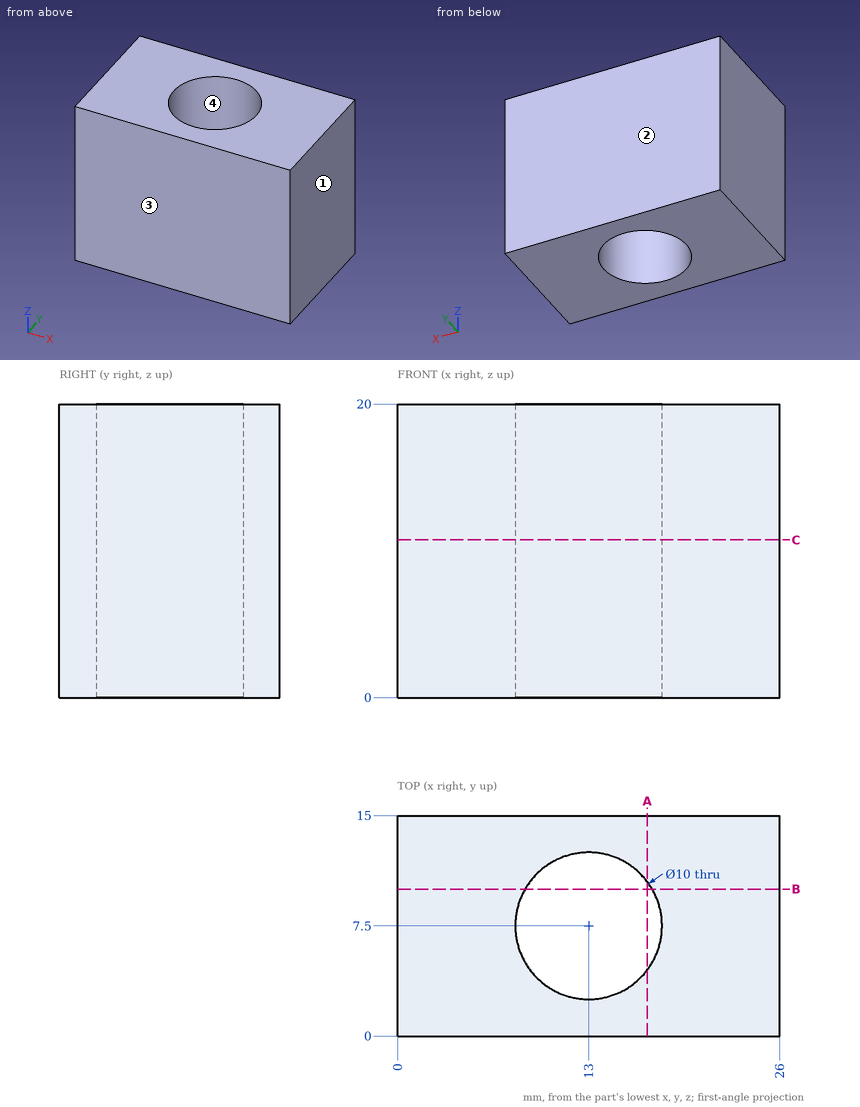
For this review, use the dimensioned drawing (mm, ordinates from the lowest corner) and the shaded views. Coordinates: 2 decimals unless noted, no trailing zeros. Loops run counter-clockwise (first coordinate to the right, second up) from the corner with the lowest first, then second, coordinate; pieces in that order, holes last. Notation, with made-up numbers: M 70,67 L 110,67 A26 ccw 110,84 Z; hole C 12.25,54 d3. An arc over 180 degrees is marked long. Answer as CSV lines item,"result".
Item 1: For probe 1 along Y at (x, z) = (13, 11.75); probe 2 along X at (y, z) = (11.25, 8); probe 3 along X at (y, z) = (9.75, 15), list the stretches that pass through material, from the lowest coordinate up.
Answer list:
probe 1,"0 to 2.5, 12.5 to 15"
probe 2,"0 to 9.69, 16.31 to 26"
probe 3,"0 to 8.53, 17.47 to 26"
Item 2: Add section C-C on z = 10.75. State the section outline as (x, y) points.
Answer list:
outline,"M 0,0 L 26,0 L 26,15 L 0,15 Z; hole C 13,7.5 d10"
Item 3: Add section A-A on x = 17. State the section outline as (y, z) points.
Answer list:
outline,"M 0,0 L 4.5,0 L 4.5,20 L 0,20 Z; M 10.5,0 L 15,0 L 15,20 L 10.5,20 Z"
Item 4: Add section B-B on y = 10. State the section outline as (x, z) points.
Answer list:
outline,"M 0,0 L 8.67,0 L 8.67,20 L 0,20 Z; M 17.33,0 L 26,0 L 26,20 L 17.33,20 Z"
Item 5: The part is to be moulded in two halves that separate along Y. For the marked faces 1, 2, 3 and 4, say which applies: pulls with the +Y half, pulls with the -Y half, needs draft (parallel to the pull), parting line crosses it, or undercut.
Answer list:
face 1,"needs draft"
face 2,"pulls with the +Y half"
face 3,"pulls with the -Y half"
face 4,"undercut"
